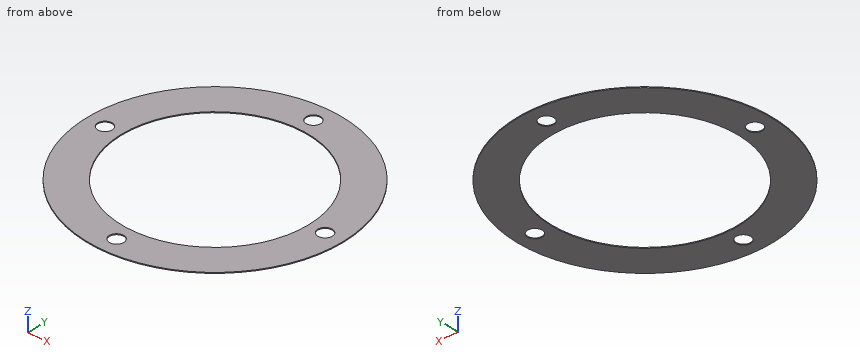
from build123d import *

# Parameters (mm, degrees)
SKETCH1_R           = 70.5
SKETCH1_R_2         = 51.5
BOSS_EXTRUDE1_DEPTH = 0.5
SKETCH2_R           = 4
CUT_EXTRUDE1_DEPTH  = 0.5


with BuildPart() as part:
    # Sketch1 → Boss-Extrude1 (new body)
    with BuildSketch(Plane.XY):
        Circle(SKETCH1_R)
        Circle(SKETCH1_R_2, mode=Mode.SUBTRACT)
    extrude(amount=BOSS_EXTRUDE1_DEPTH)

    # Sketch2 → Cut-Extrude1 (cut)
    with BuildSketch(Plane.XY.offset(0.5)):
        with Locations((0, -60.5)):
            Circle(SKETCH2_R)
        with Locations((-60.5, 0)):
            Circle(SKETCH2_R)
        with Locations((0, 60.5)):
            Circle(SKETCH2_R)
        with Locations((60.5, 0)):
            Circle(SKETCH2_R)
    extrude(amount=-CUT_EXTRUDE1_DEPTH, mode=Mode.SUBTRACT)


solid = part.part
Could you check a few things on this model? Use its own coordinates, in mm. Round coordinates to 2 decimals unless told otherwise and drop trailing zeros. Order: outer loops, then holes, each group sorted by start corner. A loop starts at its lowest first (then second) coordinate and runs counter-clockwise, first axis right, second up. Notation, with made-up numbers: M 43.5,79.25 L 81.5,79.25 A18 cw 81.5,112.25 Z; hole C 13.5,2 d5. An arc over 180 degrees is marked long. One line per item, written item: value.
(1) Imagine slicing it at C-C (z = 0.3). Write out the boundary of the cut face in (x, y).
Ans:
outline: C 0,0 d141; hole C -60.5,0 d8; hole C 0,0 d103; hole C 0,-60.5 d8; hole C 0,60.5 d8; hole C 60.5,0 d8
(2) I need wall thicknesses on line 1 along Y through (x, z) = (0, 0.3); line 2 along Y through (x, z) = (-2, 0.45); line 3 along Y through (x, z) = (5.5, 0.1). Which ranges of each line are inside material? Lowest first, please. Write a range as from..to.
Ans:
line 1: y = -70.5..-64.5, -56.5..-51.5, 51.5..56.5, 64.5..70.5
line 2: y = -70.47..-63.96, -57.04..-51.46, 51.46..57.04, 63.96..70.47
line 3: y = -70.29..-51.21, 51.21..70.29
(3) Imagine slicing it at A-A (y = 0). Write out the boundary of the cut face in (x, z), and give its area (3 significant figures).
Ans:
outline: M -70.5,0 L -64.5,0 L -64.5,0.5 L -70.5,0.5 Z; M -56.5,0 L -51.5,0 L -51.5,0.5 L -56.5,0.5 Z; M 51.5,0 L 56.5,0 L 56.5,0.5 L 51.5,0.5 Z; M 64.5,0 L 70.5,0 L 70.5,0.5 L 64.5,0.5 Z
area: 11.0 mm^2
(4) Imagine slicing it at D-D (x = 60.5). Write out the boundary of the cut face in (y, z), and give its area (3 significant figures).
Ans:
outline: M -36.19,0 L -4,0 L -4,0.5 L -36.19,0.5 Z; M 4,0 L 36.19,0 L 36.19,0.5 L 4,0.5 Z
area: 32.2 mm^2
